Source: CAD feature listing. Evaluate the final solid. Frame: model axes, mm. Round coordinates to 2 decimals unless told otherwise and drop trailing zeros. Loops run counter-clockwise (first coordinate to the right, second up) from the corner with the lowest first, then second, coordinate; pieces in that order, holes last. Notation, with made-up numbers: M -2,-32 L 49,-32 A18 ccw 49,-16 Z; hole C 53,32.25 d5. An arc over 180 degrees is marked long. Answer as a JSON object with one key per item and string values.
from build123d import *

# Parameters (mm, degrees)
SKETCH1_W           = 38
SKETCH1_H           = 22
SKETCH1_R           = 5.25
SKETCH1_R_2         = 1.75
BOSS_EXTRUDE1_DEPTH = 3
CHAMFER1_SIZE       = 1.5
CHAMFER2_SIZE       = 0.5


with BuildPart() as part:
    # Sketch1 → Boss-Extrude1 (new body)
    with BuildSketch(Plane.XY):
        Rectangle(SKETCH1_W, SKETCH1_H)
        Circle(SKETCH1_R, mode=Mode.SUBTRACT)
        with Locations((-14.5, 7.5)):
            Circle(SKETCH1_R_2, mode=Mode.SUBTRACT)
        with Locations((14.5, -7.5)):
            Circle(SKETCH1_R_2, mode=Mode.SUBTRACT)
    extrude(amount=BOSS_EXTRUDE1_DEPTH)

    # Chamfer1
    chamfer1_edges = [part.edges().sort_by_distance(p)[0] for p in [
        (19, -11, 1.5),
        (-19, -11, 1.5),
        (-19, 11, 1.5),
        (19, 11, 1.5),
    ]]
    chamfer(chamfer1_edges, length=CHAMFER1_SIZE)

    # Chamfer2
    chamfer2_edges = [part.edges().sort_by_distance(p)[0] for p in [
        (-5.25, 0, 0),
        (-5.25, 0, 3),
    ]]
    chamfer(chamfer2_edges, length=CHAMFER2_SIZE)


solid = part.part
Item 1: Section D-D on x = -14.5. Return the cut outline in (y, z).
Answer sheet:
{"outline": "M -11,0 L 5.75,0 L 5.75,3 L -11,3 Z; M 9.25,0 L 11,0 L 11,3 L 9.25,3 Z"}
Item 2: Line query: probe 1 along Y at (x, z) = (0, 1.85); probe 2 along Y at (x, z) = (14.5, 1.5); probe 3 along X at (y, z) = (8, 0.55). Output: solid intervals per line, ascending. Write a range as from..to.
Answer sheet:
{"probe 1": "y = -11..-5.25, 5.25..11", "probe 2": "y = -11..-9.25, -5.75..11", "probe 3": "x = -19..-16.18, -12.82..19"}
Item 3: Contact query for a flat-ended pin moving along its axis: pin 1 Ø5 at (x, y) = (-8, 3) entering from -Z. Output: stop coordinate, or through.
Answer sheet:
{"pin 1": "stops at z = 0"}
Item 4: Section A-A on y = 7.5. Return the cut outline in (x, z), then the cut area to 4 significant figures.
Answer sheet:
{"outline": "M -19,0 L -16.25,0 L -16.25,3 L -19,3 Z; M -12.75,0 L 19,0 L 19,3 L -12.75,3 Z", "area": "103.5 mm²"}
Item 5: Pull-direction query (Y, two-part tool) for faces 1 (the flat face through (-19, 0, 1)), 2 (the flat face through (18.3, -10.2, 1.5)), 3 (the cylindrical face through (-12.883, 6.83, 1.479)); classes: pulls with the +Y half, pulls with the -Y half, needs draft (parallel to the pull), parting line crosses it, or undercut.
Answer sheet:
{"face 1": "needs draft", "face 2": "pulls with the -Y half", "face 3": "undercut"}
Item 6: Section B-B on x = 0. Return the cut outline in (y, z), then the cut area to 3 significant figures.
Answer sheet:
{"outline": "M -11,0 L -5.75,0 L -5.25,0.5 L -5.25,2.5 L -5.75,3 L -11,3 Z; M 5.25,0.5 L 5.75,0 L 11,0 L 11,3 L 5.75,3 L 5.25,2.5 Z", "area": "34.0 mm²"}
Item 7: Section C-C on z = 1.4. Return the cut outline in (x, y).
Answer sheet:
{"outline": "M -19,-9.5 L -17.5,-11 L 17.5,-11 L 19,-9.5 L 19,9.5 L 17.5,11 L -17.5,11 L -19,9.5 Z; hole C -14.5,7.5 d3.5; hole C 0,0 d10.5; hole C 14.5,-7.5 d3.5"}
